For this review, take the finished solid that the model builds, in its own axes (mm). Face numbers are marked on the shaded views. A direction names the side the tool comes from. Give positions to 0.01 mm unless a question says otherwise; leave off trailing zeros. Order: outer loops, then holes, each group sorted by start corner. A loop starts at its lowest first (then second) coordinate and runs counter-clockwise, first axis right, second up. Notation, with made-up numbers: (60, -5) - (118, -5) arc R33 ccw to (118, 23) - close; hole circle Ø8 at (-19, 62). An arc over 180 degrees is marked (long way). Put each result on its own line as item: value. Start each with the question number.
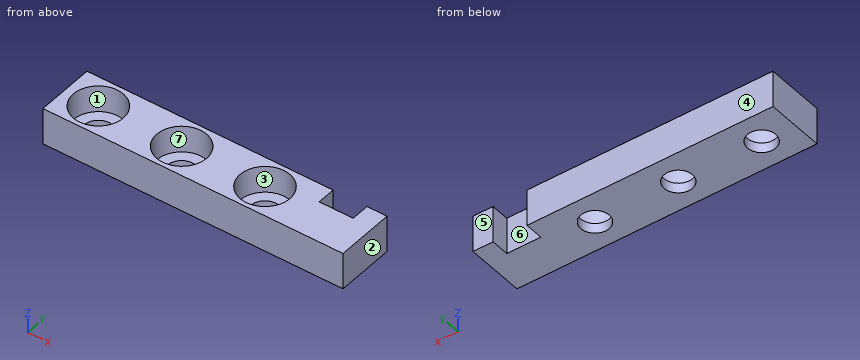
```python
from build123d import *

# Parameters (mm, degrees)
SKETCH1_R           = 4.25
BOSS_EXTRUDE1_DEPTH = 11
SKETCH2_R           = 7.5
CUT_EXTRUDE1_DEPTH  = 8


with BuildPart() as part:
    # Sketch1 → Boss-Extrude1 (new body)
    with BuildSketch(Plane.XY):
        Polygon((-45, 8.75), (28.8, 8.75), (28.8, 3.25), (39, 3.25), (39, 8.75), (45, 8.75), (45, -8.75), (-45, -8.75), align=None)
        with Locations((-35, 0)):
            Circle(SKETCH1_R, mode=Mode.SUBTRACT)
        with Locations((-10, 0)):
            Circle(SKETCH1_R, mode=Mode.SUBTRACT)
        with Locations((15, 0)):
            Circle(SKETCH1_R, mode=Mode.SUBTRACT)
    extrude(amount=BOSS_EXTRUDE1_DEPTH)

    # Sketch2 → Cut-Extrude1 (cut)
    with BuildSketch(Plane.XY.offset(11)):
        with Locations((-35, 0)):
            Circle(SKETCH2_R)
        with Locations((-10, 0)):
            Circle(SKETCH2_R)
        with Locations((15, 0)):
            Circle(SKETCH2_R)
    extrude(amount=-CUT_EXTRUDE1_DEPTH, mode=Mode.SUBTRACT)


solid = part.part
```
1. Add section D-D, the plane y = -6. Give the boundary of the cut face in (x, z), then the cut area to 3 significant figures.
2. The part is to be moulded in two halves that separate along X. For the marked faces 1, 2, 3 and 4, say which applies: released by +X, released by -X, zero draft, split by the parting line, or undercut.
3. Clearance check with flat-ended pins moving along their axes: pin 1 (2 mm diameter, centred on x = 27, y = -1.5, fed in from -Z); pin 2 (7.5 mm diameter, centred on x = 14.5, y = 1.5, fed in from +Z); pin 3 (5 mm diameter, centred on x = 15, y = 0, fed in from +Z). State where each tip first meets the part, or that it passes through.
4. Add section C-C, the plane x = -35. Give the boundary of the cut face in (y, z).
5. Tool access review of the marked faces 5, 6 and 7: name each direction out of +Z, -Z, +X, -X, +Y, -Y from which nothing blocks a thin tool from reaching the whole face with its end or side.
6. Wall thickness on line 1 (X direction, y = 0, z = 1.9); line 2 (X direction, y = 6.75, z = 6); line 3 (Y direction, x = -10, z = 5.75): over which ranges is each line inside the solid? List them lowest first. Write a range as from..to.
7. Add section A-A, the plane y = 0. Give the boundary of the cut face in (x, z), then the cut area to 4 significant figures.
8. Add section B-B, the plane z = 5.25. Give the boundary of the cut face in (x, y), then the cut area to 3 significant figures.
Found:
1. outline: (-45, 0) - (45, 0) - (45, 11) - (19.5, 11) - (19.5, 3) - (10.5, 3) - (10.5, 11) - (-5.5, 11) - (-5.5, 3) - (-14.5, 3) - (-14.5, 11) - (-30.5, 11) - (-30.5, 3) - (-39.5, 3) - (-39.5, 11) - (-45, 11) - close
1. area: 774 mm^2
2. face 1: undercut
2. face 2: released by +X
2. face 3: undercut
2. face 4: zero draft
3. pin 1: stops at z = 0
3. pin 2: stops at z = 3
3. pin 3: passes through
4. outline: (-8.75, 0) - (-4.25, 0) - (-4.25, 3) - (-7.5, 3) - (-7.5, 11) - (-8.75, 11) - close; (4.25, 0) - (8.75, 0) - (8.75, 11) - (7.5, 11) - (7.5, 3) - (4.25, 3) - close
5. face 5: +Z, -Z, +X, -X, +Y
5. face 6: +Z, -Z, +Y
5. face 7: +Z
6. line 1: x = -45..-39.25, -30.75..-14.25, -5.75..10.75, 19.25..45
6. line 2: x = -45..-38.27, -31.73..-13.27, -6.73..11.73, 18.27..28.8, 39..45
6. line 3: y = -8.75..-7.5, 7.5..8.75
7. outline: (-45, 0) - (-39.25, 0) - (-39.25, 3) - (-42.5, 3) - (-42.5, 11) - (-45, 11) - close; (-30.75, 0) - (-14.25, 0) - (-14.25, 3) - (-17.5, 3) - (-17.5, 11) - (-27.5, 11) - (-27.5, 3) - (-30.75, 3) - close; (-5.75, 0) - (10.75, 0) - (10.75, 3) - (7.5, 3) - (7.5, 11) - (-2.5, 11) - (-2.5, 3) - (-5.75, 3) - close; (19.25, 0) - (45, 0) - (45, 11) - (22.5, 11) - (22.5, 3) - (19.25, 3) - close
7. area: 553.5 mm^2
8. outline: (-45, -8.75) - (45, -8.75) - (45, 8.75) - (39, 8.75) - (39, 3.25) - (28.8, 3.25) - (28.8, 8.75) - (-45, 8.75) - close; hole circle Ø15 at (-35, 0); hole circle Ø15 at (-10, 0); hole circle Ø15 at (15, 0)
8. area: 989 mm^2
